```python
from build123d import *

# Parameters (mm, degrees)
BOSS_EXTRUDE1_DEPTH                     = 460
CBORE_FOR_M8_HEX_HEAD_BOLT1_D           = 9
CBORE_FOR_M8_HEX_HEAD_BOLT1_CBORE_D     = 18
CBORE_FOR_M8_HEX_HEAD_BOLT1_CBORE_DEPTH = 10
M8_TAPPED_HOLE1_D                       = 6.8
M8_TAPPED_HOLE1_DEPTH                   = 19.75
M8_TAPPED_HOLE1_TIP                     = 2.042926105


with BuildPart() as part:
    # Sketch1 → Boss-Extrude1 (new body)
    with BuildSketch(Plane.XY):
        Polygon((-40, 52.5), (-40, 55.5), (40, 55.5), (40, 52.5), (70, 52.5), (71.711448084, 53.534864946), (73.263745503, 50.96769282), (69.385770597, 48.622789502), (48, 18.080743852), (48, 12.5), (100, 12.5), (100, 67.5), (-100, 67.5), (-100, 12.5), (-48, 12.5), (-48, 18.080743852), (-69.385770597, 48.622789502), (-73.263745503, 50.96769282), (-71.711448084, 53.534864946), (-70, 52.5), align=None)
    extrude(amount=-BOSS_EXTRUDE1_DEPTH)

    # CBORE for M8 Hex Head Bolt1 (through all)
    with Locations(Plane(origin=(0, 67.5, 0), x_dir=(1, 0, 0), z_dir=(0, 1, 0))):
        with Locations((0, 247.5), (0, 212.5)):
            CounterBoreHole(CBORE_FOR_M8_HEX_HEAD_BOLT1_D / 2, CBORE_FOR_M8_HEX_HEAD_BOLT1_CBORE_D / 2, CBORE_FOR_M8_HEX_HEAD_BOLT1_CBORE_DEPTH)

    # M8 Tapped Hole1
    with Locations(Plane(origin=(0, 67.5, 0), x_dir=(1, 0, 0), z_dir=(0, 1, 0))):
        with Locations((1.4e-07, 230), (80.000000279, 430), (-80, 30), (-80, 430), (80.000000279, 30), (-80, 350), (80.000000279, 350), (-80, 270), (80.000000279, 270), (-80, 190), (80.000000279, 190), (-80, 110), (80.000000279, 110)):
            Hole(M8_TAPPED_HOLE1_D / 2, depth=M8_TAPPED_HOLE1_DEPTH)
            with Locations((0, 0, -(M8_TAPPED_HOLE1_DEPTH + M8_TAPPED_HOLE1_TIP / 2))):  # 118° drill point
                Cone(0, M8_TAPPED_HOLE1_D / 2, M8_TAPPED_HOLE1_TIP, mode=Mode.SUBTRACT)


solid = part.part
```
The listing builds one solid part. Answer for the finished solid, in the listing's coordinates (mm). A direction names the side the tool comes from. Coordinates: 2 decimals unless noted, no trailing zeros. Loops run counter-clockwise (first coordinate to the right, second up) from the corner with the lowest first, then second, coordinate; pieces in that order, holes last. Notation, with made-up numbers: M 44.25,55 L 54.25,55 A22 cw 54.25,76 Z; hole C 34,82 d10. An arc over 180 degrees is marked long. Answer as a JSON object with one key per item and string values. Group by question number.
Item 1: Determine the mould class of faces 1 (the face through (-1, 59, -460)), 2 (the face through (8, 55.5, -227)), 3 (the face through (0.98, 56.49, -243.11)), 4 (the face through (-1.172, 62.57, -221.423)) for opening direction Z: +Z half, -Z half, draft (parallel to the pull), parting line (faces both ways), or undercut.
Item 2: Which of the six approach directions +Z, -Z, +X, -X, +Y, -Y give full straight-line access (tool end or side, diameter ignored) to faces 5 (the face through (2, 57.5, -252)), 6 (the face through (-100, 40, -227)), 7 (the face through (-55, 52.5, -227))?
Item 3: Section C-C (y = 38) is taken. Write down the section's boundary in (x, z), and give its area (3 significant figures).
Item 4: Each of these flat-tipped pins is pushed along its axis until it touches: P1, Ø6, axis at x = -80, z = -350, coming from the +Y side; P2, Ø1, axis at x = 11, z = -119.5, coming from the -Y side; P3, Ø10.5, axis at x = 0, z = -212.5, coming from the +Y side. Where does it stop, or does it pass through?
Item 5: Section A-A (x = -56.5) is taken. Write down the section's boundary in (y, z).
Item 6: Section B-B (z = -212.5) is taken. Write down the section's boundary in (x, y).
Item 7: Section D-D (z = -363.5) is taken. Write down the section's boundary in (x, y), and give its area (3 significant figures).
Item 8: Consider L1, parallel to X at y = 58.25, z = -430; L2, parallel to X at y = 63, z = -32; L3, parallel to X at y = 49, z = -253. Determine where each line is inside the solid, lowest interval first.
Solved:
{
 "1": {"face 1": "-Z half", "face 2": "draft", "face 3": "undercut", "face 4": "undercut"},
 "2": {"face 5": "+Y", "face 6": "+Z, -Z, -X, +Y, -Y", "face 7": "+Z, -Z"},
 "3": {"outline": "M -100,-460 L -61.95,-460 L -61.95,0 L -100,0 Z; M 61.95,-460 L 100,-460 L 100,0 L 61.95,0 Z", "area": "35,000 mm2"},
 "4": {"P1": "stops at y = 47.51", "P2": "stops at y = 55.5", "P3": "stops at y = 57.5"},
 "5": {"outline": "M 12.5,-460 L 30.22,-460 L 30.22,0 L 12.5,0 Z; M 52.5,-460 L 67.5,-460 L 67.5,0 L 52.5,0 Z"},
 "6": {"outline": "M -100,12.5 L -48,12.5 L -48,18.08 L -69.39,48.62 L -73.26,50.97 L -71.71,53.53 L -70,52.5 L -40,52.5 L -40,55.5 L -4.5,55.5 L -4.5,57.5 L -9,57.5 L -9,67.5 L -100,67.5 Z; M 4.5,55.5 L 40,55.5 L 40,52.5 L 70,52.5 L 71.71,53.53 L 73.26,50.97 L 69.39,48.62 L 48,18.08 L 48,12.5 L 100,12.5 L 100,67.5 L 9,67.5 L 9,57.5 L 4.5,57.5 Z"},
 "7": {"outline": "M -100,12.5 L -48,12.5 L -48,18.08 L -69.39,48.62 L -73.26,50.97 L -71.71,53.53 L -70,52.5 L -40,52.5 L -40,55.5 L 40,55.5 L 40,52.5 L 70,52.5 L 71.71,53.53 L 73.26,50.97 L 69.39,48.62 L 48,18.08 L 48,12.5 L 100,12.5 L 100,67.5 L -100,67.5 Z", "area": "6,080 mm2"},
 "8": {"L1": "x = -100 to -83.4, -76.6 to 76.6, 83.4 to 100", "L2": "x = -100 to -82.75, -77.25 to 77.25, 82.75 to 100", "L3": "x = -100 to -70.01, 70.01 to 100"}
}
